```python
from build123d import *

# Parameters (mm, degrees)
M3_TAPPED_HOLE1_D     = 2.5
M3_TAPPED_HOLE1_DEPTH = 10
M3_TAPPED_HOLE1_TIP   = 0.751075774
FILLET1_R             = 2


with BuildPart() as part:
    # Sketch1 → Revolve1 (revolve)
    with BuildSketch(Plane.XY):
        Polygon((0, 0), (0, 15), (2.5, 15), (4, 12), (4, 3), (3, 3), (3, 0), align=None)
    revolve(axis=Axis((0, 0, 0), (0, 1, 0)))

    # M3 Tapped Hole1
    with Locations(Plane(origin=(0, 0, 0), x_dir=(-1, 0, 0), z_dir=(0, -1, 0))):
        with Locations((0, 0)):
            Hole(M3_TAPPED_HOLE1_D / 2, depth=M3_TAPPED_HOLE1_DEPTH)
            with Locations((0, 0, -(M3_TAPPED_HOLE1_DEPTH + M3_TAPPED_HOLE1_TIP / 2))):  # 118° drill point
                Cone(0, M3_TAPPED_HOLE1_D / 2, M3_TAPPED_HOLE1_TIP, mode=Mode.SUBTRACT)

    # Fillet1
    fillet1_edges = [part.edges().sort_by_distance(p)[0] for p in [
        (-4, 12, 0),
    ]]
    fillet(fillet1_edges, radius=FILLET1_R)


solid = part.part
```
Work out the finished part from the listing and answer in its coordinate system (mm). A direction names the side the tool comes from. Round coordinates to 2 decimals unless told otherwise and drop trailing zeros. Loops run counter-clockwise (first coordinate to the right, second up) from the corner with the lowest first, then second, coordinate; pieces in that order, holes last.
(1) Each of these flat-tipped pins is pushed along its axis until it touches: P1, Ø1.5, axis at x = 1.5, y = 2, coming from the -Z side; P2, Ø2, axis at x = 1.5, y = 3, coming from the +Z side; P3, Ø1.5, axis at y = 11, z = 2.5, coming from the -X side; P4, Ø1.5, axis at x = 1, z = 0.5, coming from the -Y side. Where does it stop, or does it pass through?
Computed values:
P1: stops at z = -2.9
P2: stops at z = 3.97
P3: stops at x = -3.6
P4: stops at y = 0
(2) The part is cut by section A-A, the plane y = 6.5. Give the vertices of the cut face in (x, z).
Computed values:
outline: circle Ø8 at (0, 0); hole circle Ø2.5 at (0, 0)
(3) For faces 4 (the conical face through (2.46, 14.84, -0.78)), 5 (the cylindrical face through (-3, 1, 0)), determine the directions among +Z, -Z, +X, -X, +Y, -Y from which every point of the face is accessible in a straight line to the end or side of a thin tool.
Computed values:
face 4: +Y
face 5: -Y
(4) Find the intervals of material crossed by L1, parallel to Z at x = 0, y = 2.5; L2, parallel to Z at x = 0, y = 7.75; L3, parallel to X at y = 8.75, z = -1, in increasing order.
Computed values:
L1: z = -3 to -1.25, 1.25 to 3
L2: z = -4 to -1.25, 1.25 to 4
L3: x = -3.87 to -0.75, 0.75 to 3.87
(5) The mould has two halves that part along X. Classify faces 1 (the flat face through (1, 3, -3)), 2 (the cylindrical face through (3.695, 7.204, 1.532)), 3 (the conical face through (0.05, 10.62, 0.21)): pulls with the +X half, pulls with the -X half, needs draft (parallel to the pull), parting line crosses it, or undercut.
Computed values:
face 1: needs draft
face 2: parting line crosses it
face 3: undercut
